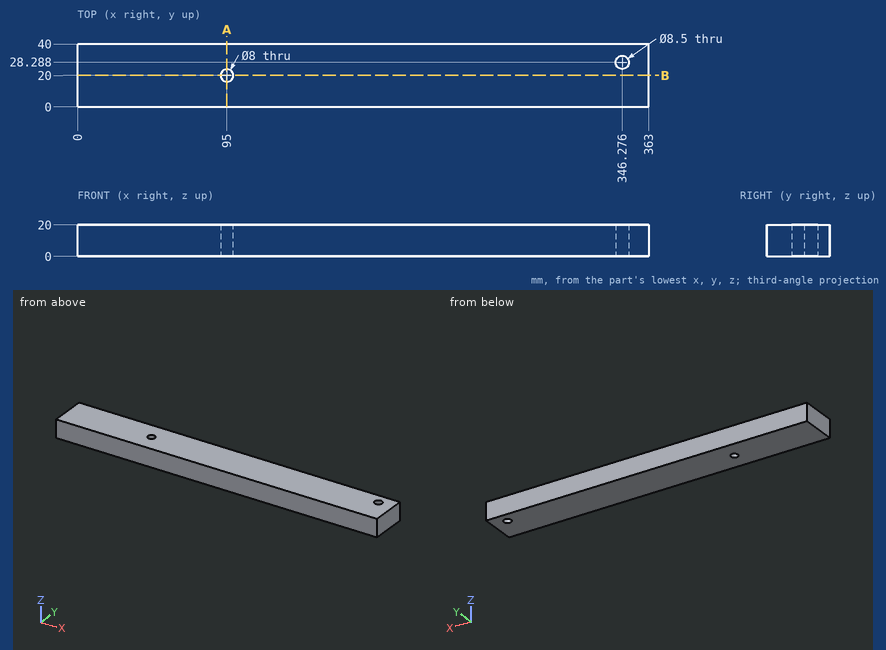
The figure shows three views and two pictorial views of one solid part (mm, origin at its lowest corner). Answer the questions. Coordinates: 2 decimals unless noted, no trailing zeros. Loops run counter-clockwise (first coordinate to the right, second up) from the corner with the lowest first, then second, coordinate; pieces in that order, holes last. Notation, with made-up numbers: (29.25, 10.25) -> (50.25, 10.25) arc R16 ccw to (50.25, 24.25) -> close; hole circle Ø7 at (-17.5, 11). An arc over 180 degrees is marked (long way). Use one line per item in the form item = value. Start each with the question number.
Item 1: Consider L1, parallel to X at y = 27.5, z = 11.25; L2, parallel to Y at x = 95, z = 13.75; L3, parallel to X at y = 23.5, z = 11.25. Determine where each line is inside the solid, lowest interval first. Write a range as [from, to].
Item 2: The part is cut by section A-A on x = 95. Determine the outline of the cut face in (y, z), then the cut area to 3 significant figures.
Item 3: The part is cut by section B-B on y = 20. Determine the outline of the cut face in (x, z), then the cut area to 3 significant figures.
Item 4: A flat-ended cylindrical pin translates along its axis: pin 1 Ø1.5 at (y, z) = (9.5, 16.5) entering from -X. Find the tip coordinate at first contact, or state that the pin passes through.
Answer key:
q1.L1 = [0, 342.1], [350.45, 363]
q1.L2 = [0, 16], [24, 40]
q1.L3 = [0, 93.06], [96.94, 363]
q2.outline = (0, 0) -> (16, 0) -> (16, 20) -> (0, 20) -> close; (24, 0) -> (40, 0) -> (40, 20) -> (24, 20) -> close
q2.area = 640 mm2
q3.outline = (0, 0) -> (91, 0) -> (91, 20) -> (0, 20) -> close; (99, 0) -> (363, 0) -> (363, 20) -> (99, 20) -> close
q3.area = 7,100 mm2
q4.pin_1 = 0
